For this review, take the finished solid that the model builds, in its own axes (mm). A direction names the side the tool comes from. Give positions to 0.01 mm unless a question says otherwise; leave off trailing zeros. Order: outer loops, then holes, each group sorted by start corner. A loop starts at its lowest first (then second) coordinate and runs counter-clockwise, first axis right, second up.
Item 1: Consider section B-B (y = 93.5). Give the boundary of the cut face in (x, z), plus the area to 3 significant figures.
Item 2: Machinability: for faces 1 (the flat face through (319, 178, 2)), 2 (the cylindrical face through (181.486, 5.703, -2.1)), 3 (the cylindrical face through (-4.95, 69.02, 112.39)), 4 (the flat face through (-316, 178, 2)), which of the approach directions +Z, -Z, +X, -X, +Y, -Y give a long, thin tool a straight path to every point of the face, cutting with its end or side? Answer none if there is none.
Item 3: Consider section C-C (x = 355). Give the boundary of the cut face in (y, z), plus the area to 3 significant figures.
Item 4: Consider section A-A (y = 188). Give the boundary of the cut face in (x, z), plus the area to 3 significant figures.
Item 5: The part is to be moulded in two halves that separate along X. For faces 5 (the flat face through (-301, 208, 2)), 6 (the flat face through (-114, 0, 2)), 7 (the flat face through (475, 193, 2)), say which applies: released by +X, released by -X, zero draft, split by the parting line, or undercut.
Item 6: Consider section D-D (z = 127.5). Give the boundary of the cut face in (x, y).
Item 7: For P1, Ø12, axis at y = 118, z = 119.5, coming from the -X side; P2, Ø3, axis at x = -277, z = 76.5, coming from the -Y side; P3, Ø5, axis at x = 40, z = -95, coming from the +Y side, all flat-tipped, find the tip position at first contact; note any pin that passes through.
Item 8: For probe 1 along X at (y, z) = (187, 0); probe 2 along X at (y, z) = (46, 0); probe 3 along X at (y, z) = (141, 40), list the stretches that pass through material, from the lowest coordinate up.
```python
from build123d import *

# Parameters (mm, degrees)
Z_BRACKET_BODY_DEPTH        = 150
TUBE_BOSS_SKETCH_R          = 112.5
TUBE_BOSS_SKETCH_R_2        = 87.5
TUBE_BOSS_225X_175_DEPTH    = 140
CENTRE_HOLE_SKETCH_R        = 37.5
CENTRE_HOLE_75_DEPTH        = 140
FLANGE_HOLES_SKETCH_R       = 25
FLANGE_MOUNTING_HOLES_DEPTH = 140
BEND_FILLET_R20_R           = 20
BEND_FILLET_R50_R           = 50


with BuildPart() as part:
    # Bracket Profile Sketch → Z Bracket Body (new, symmetric)
    with BuildSketch(Plane.XY):
        Polygon((-475, 208), (-187.5, 208), (-187.5, 0), (187.5, 0), (187.5, 208), (475, 208), (475, 178), (217.5, 178), (217.5, -30), (-217.5, -30), (-217.5, 178), (-475, 178), align=None)
    extrude(amount=Z_BRACKET_BODY_DEPTH, both=True)

    # Tube Boss Sketch → Tube Boss Ø225xØ175 (add)
    with BuildSketch(Plane(origin=(0, 0, 0), x_dir=(1, 0, 0), z_dir=(0, 1, 0))):
        with Locations(Location((0, 0, 0), (0, 0, 90))):
            Circle(TUBE_BOSS_SKETCH_R)
        with Locations(Location((0, 0, 0), (0, 0, 270))):
            Circle(TUBE_BOSS_SKETCH_R_2, mode=Mode.SUBTRACT)
    extrude(amount=TUBE_BOSS_225X_175_DEPTH)

    # Centre Hole Sketch → Centre Hole Ø75 (cut)
    with BuildSketch(Plane(origin=(0, 0, 0), x_dir=(1, 0, 0), z_dir=(0, 1, 0))):
        with Locations(Location((0, 0, 0), (0, 0, 270))):
            Circle(CENTRE_HOLE_SKETCH_R)
    extrude(amount=-CENTRE_HOLE_75_DEPTH, mode=Mode.SUBTRACT)

    # Flange Holes Sketch → Flange Mounting Holes (cut)
    with BuildSketch(Plane(origin=(0, 208, 0), x_dir=(1, 0, 0), z_dir=(0, 1, 0))):
        with Locations(Location((-355, 0, 0), (0, 0, 270))):
            Circle(FLANGE_HOLES_SKETCH_R)
        with Locations(Location((355, 0, 0), (0, 0, 270))):
            Circle(FLANGE_HOLES_SKETCH_R)
    extrude(amount=-FLANGE_MOUNTING_HOLES_DEPTH, mode=Mode.SUBTRACT)

    # Bend Fillet R20
    bend_fillet_r20_edges = [part.edges().sort_by_distance(p)[0] for p in [
        (-187.5, 0, 0),
        (187.5, 0, 0),
    ]]
    fillet(bend_fillet_r20_edges, radius=BEND_FILLET_R20_R)

    # Bend Fillet R50
    bend_fillet_r50_edges = [part.edges().sort_by_distance(p)[0] for p in [
        (217.5, -30, 0),
        (-217.5, -30, 0),
    ]]
    fillet(bend_fillet_r50_edges, radius=BEND_FILLET_R50_R)


solid = part.part
```
Resolved:
1. outline: (-217.5, -150) - (-187.5, -150) - (-187.5, 150) - (-217.5, 150) - close; circle Ø225 at (0, 0); (187.5, -150) - (217.5, -150) - (217.5, 150) - (187.5, 150) - close; hole circle Ø175 at (0, 0)
1. area: 33,700 mm2
2. face 1: +Z, -Z, +X, -Y
2. face 2: +Z, -Z, +Y
2. face 3: +Y
2. face 4: +Z, -Z, -X, -Y
3. outline: (178, -150) - (208, -150) - (208, -25) - (178, -25) - close; (178, 25) - (208, 25) - (208, 150) - (178, 150) - close
3. area: 7,500 mm2
4. outline: (-475, -150) - (-187.5, -150) - (-187.5, 150) - (-475, 150) - close; (187.5, -150) - (475, -150) - (475, 150) - (187.5, 150) - close; hole circle Ø50 at (-355, 0); hole circle Ø50 at (355, 0)
4. area: 169,000 mm2
5. face 5: zero draft
5. face 6: undercut
5. face 7: released by +X
6. outline: (-475, 178) - (-217.5, 178) - (-217.5, 20) arc R50 ccw to (-167.5, -30) - (167.5, -30) arc R50 ccw to (217.5, 20) - (217.5, 178) - (475, 178) - (475, 208) - (187.5, 208) - (187.5, 20) arc R20 cw to (167.5, 0) - (-167.5, 0) arc R20 cw to (-187.5, 20) - (-187.5, 208) - (-475, 208) - close
7. P1: stops at x = -217.5
7. P2: stops at y = 178
7. P3: stops at y = 140
8. probe 1: x = -475 to -380, -330 to -187.5, 187.5 to 330, 380 to 475
8. probe 2: x = -217.5 to -187.5, -112.5 to -87.5, 87.5 to 112.5, 187.5 to 217.5
8. probe 3: x = -217.5 to -187.5, 187.5 to 217.5
